```python
from build123d import *

# Parameters (mm, degrees)
SKETCH1_R           = 38.1
BOSS_EXTRUDE1_DEPTH = 4


with BuildPart() as part:
    # Sketch1 → Boss-Extrude1 (new, symmetric)
    with BuildSketch(Plane.XY):
        with BuildLine():
            Line((1000.125, 641.35), (1000.125, -45.0629))
            Line((1000.125, -45.0629), (1215.934413963, -617.113829271))
            ThreePointArc((1215.934413963, -617.113829271), (1256.96824156, -683.459757951), (1319.975225131, -729.45625))
            ThreePointArc((1319.975225131, -729.45625), (1507.976686944, -21.150112495), (1339.913949896, 692.15))
            Line((1339.913949896, 692.15), (1336.870808151, 690.572164727))
            ThreePointArc((1336.870808151, 690.572164727), (1310.307279769, 726.359551875), (1273.824497124, 751.959643467))
            Line((1273.824497124, 751.959643467), (1153.31875, 810.41875))
            Line((1153.31875, 810.41875), (1015.69584463, 677.949817102))
            ThreePointArc((1015.69584463, 677.949817102), (1004.179513091, 661.237168064), (1000.125, 641.35))
        make_face()
        with Locations((1228.725, 663.575)):
            Circle(SKETCH1_R, mode=Mode.SUBTRACT)
    extrude(amount=BOSS_EXTRUDE1_DEPTH, both=True)


solid = part.part
```
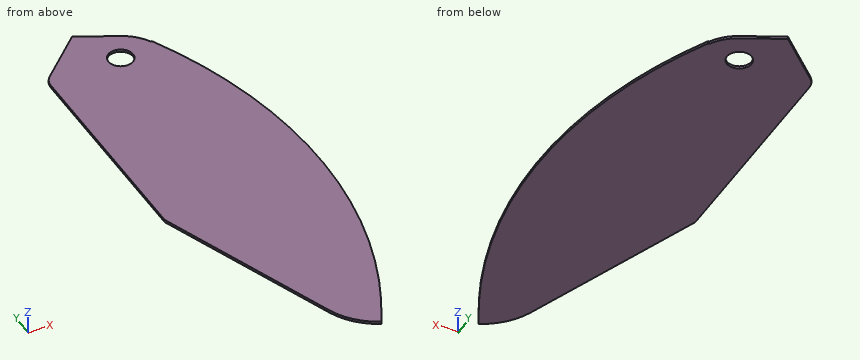
Source: CAD feature listing. Evaluate the final solid. Frame: model axes, mm. Give positions to 0.01 mm unless a question says otherwise; leave off trailing zeros. Loops run counter-clockwise (first coordinate to the right, second up) from the corner with the lowest first, then second, coordinate; pieces in that order, holes last. Notation, with made-up numbers: (87.25, 30) - (117.25, 30) arc R31 cw to (117.25, 62) - close; hole circle Ø10 at (-38, -31.75). An arc over 180 degrees is marked (long way). Use CSV: the item, a comma, the result in double quotes. Start each with the question number.
1. Section C-C (y = 443.5). Output: boundary loops of the cut face in (x, z) (3 decimals), then the cut area to 3 significant figures.
2. Section B-B (x = 1394.5). Output: boundary loops of the cut face in (y, z), then the cut area to 3 significant figures.
3. Ray query, L1, parallel to Y at x = 1218.5, z = 1; L2, parallel to Y at x = 1319, z = -2.25; L3, parallel to X at y = 85, z = 2.5 (3 decimals). Return the intervals inside material, ascending.
4. Pin query (flat end, axial travel): pin 1 (2 mm diameter, centred on y = -151, z = -1.5, fed in from +X); pin 2 (2 mm diameter, centred on x = 1293, z = 1.5, fed in from -Y). Return the tip coordinate at first contact, or that it passes through.
Response:
1,outline,"(1000.125, -4) - (1441.44, -4) - (1441.44, 4) - (1000.125, 4) - close"
1,area,"3,530 mm²"
2,outline,"(-574.29, -4) - (574.29, -4) - (574.29, 4) - (-574.29, 4) - close"
2,area,"9,190 mm²"
3,L1,"-623.58 to 626.87, 700.28 to 778.8"
3,L2,"-729 to 717.09"
3,L3,"1000.125 to 1505.728"
4,pin 1,"x = 1500.65"
4,pin 2,"y = -714.9"
